```python
from build123d import *

# Parameters (mm, degrees)
BASE_BLOCK_SKETCH_W   = 70
BASE_BLOCK_SKETCH_H   = 30
BASE_BLOCK_DEPTH      = 20
HINGE_EAR_SKETCH_R    = 5
HINGE_EAR_DEPTH       = 10
SIDE_BLOCK_SKETCH_W   = 10
SIDE_BLOCK_SKETCH_H   = 10
SIDE_BLOCK_DEPTH      = 10
STOP_BLOCK_SKETCH_W   = 10
STOP_BLOCK_SKETCH_H   = 10
STOP_BLOCK_10MM_DEPTH = 10
ROD_SKETCH_R          = 2.5
ROD_30MM_DEPTH        = 30


with BuildPart() as part:
    # Base Block Sketch → Base Block (new body)
    with BuildSketch(Plane.XY):
        with Locations((35, 15)):
            Rectangle(BASE_BLOCK_SKETCH_W, BASE_BLOCK_SKETCH_H)
    extrude(amount=BASE_BLOCK_DEPTH)

    # Hinge Ear Sketch → Hinge Ear (add)
    with BuildSketch(Plane(origin=(0, 0, 0), x_dir=(0, 0, -1), z_dir=(1, 0, 0))):
        with BuildLine():
            Line((-20, 40), (-20, 30))
            Line((-20, 30), (0, 30))
            Line((0, 30), (0, 40))
            ThreePointArc((0, 40), (-10, 50), (-20, 40))
        make_face()
        with Locations((-10, 40)):
            Circle(HINGE_EAR_SKETCH_R, mode=Mode.SUBTRACT)
    hinge_ear = extrude(amount=HINGE_EAR_DEPTH)

    # Hinge Ear Mirror: Hinge Ear across plane
    add(hinge_ear.mirror(Plane(origin=(35, 0, 0), x_dir=(0, 0, 1), z_dir=(1, 0, 0))))

    # Side Block Sketch → Side Block (add)
    with BuildSketch(Plane.XY.offset(20)):
        with Locations((55, 15)):
            Rectangle(SIDE_BLOCK_SKETCH_W, SIDE_BLOCK_SKETCH_H)
    side_block = extrude(amount=SIDE_BLOCK_DEPTH)

    # Stop Block Sketch → Stop Block 10mm (add)
    with BuildSketch(Plane.XY.offset(20)):
        with Locations((15, 15)):
            Rectangle(STOP_BLOCK_SKETCH_W, STOP_BLOCK_SKETCH_H)
    stop_block_10mm = extrude(amount=STOP_BLOCK_10MM_DEPTH)

    # Rod Sketch → Rod 30mm (add)
    with BuildSketch(Plane(origin=(20, 0, 0), x_dir=(0, 0, -1), z_dir=(1, 0, 0))):
        with Locations(Location((-25, 15, 0), (0, 0, 180))):
            Circle(ROD_SKETCH_R)
    rod_30mm = extrude(amount=ROD_30MM_DEPTH)

    # Block and Rod Mirror: Side Block, Stop Block 10mm, Rod 30mm across plane
    add(side_block.mirror(Plane.XY.offset(10)))
    add(stop_block_10mm.mirror(Plane.XY.offset(10)))
    add(rod_30mm.mirror(Plane.XY.offset(10)))


solid = part.part
```
The model under review builds one solid part; all positions refer to its coordinate system, in mm. A direction names the side the tool comes from. Coordinates: 2 decimals unless noted, no trailing zeros. Order: outer loops, then holes, each group sorted by start corner. A loop starts at its lowest first (then second) coordinate and runs counter-clockwise, first axis right, second up. Notation, with made-up numbers: (35, -16) -> (44, -16) arc R25 ccw to (44, 17) -> close; hole circle Ø6 at (81, -33.75). An arc over 180 degrees is marked (long way). Answer in a Markdown table with one row per item. Add a question column.
Item 1: We need section B-B on x = 42. Write out the cut boundary in (y, z).
Item 2: Mouldability with a two-part tool opening along Z and no side actions: class faces 6 (the flat face through (55, 15, -10)), 7 (the cylindrical face through (5, 44, 7)), 8 (the flat face through (60, 38, 15)) as +Z half, -Z half, draft (parallel to the pull), parting line (faces both ways), or undercut.
Item 3: Machinability: for faces 1 (the flat face through (15, 20, 25)), 2 (the flat face through (60, 15, 25)), 3 (the flat face through (60, 15, -5)), 4 (the flat face through (55, 20, -5)), 5 (the flat face through (10, 15, 25)), which of the approach directions +Z, -Z, +X, -X, +Y, -Y give a long, thin tool a straight path to every point of the face, cutting with its end or side? Answer none if there is none.
Item 4: We need section D-D on y = 15. Write out the cut boundary in (x, z).
Item 5: We need section C-C on z = 10. Write out the cut boundary in (x, y).
Item 6: Clearance check with flat-ended pins moving along their axes: pin 1 (3 mm diameter, centred on x = 36.5, y = 6, fed in from -Z); pin 2 (2 mm diameter, centred on x = 50, y = 8, fed in from +Z); pin 3 (5 mm diameter, centred on x = 52.5, z = 24.5, fed in from +Y). State where each tip first meets the part, or that it passes through.
Item 7: To check wall thickness, follow probe 1 along Z at (x, y) = (22.5, 15); probe 2 along Y at (x, z) = (66, 10); probe 3 along X at (y, z) = (11.5, -6.5). State the ranges of each line that lie inside material, in increasing order.
Item 8: We need section A-A on z = 21.5. Write out the cut boundary in (x, y), plus the area to 3 significant figures.
Final values:
| question | item | result |
|---|---|---|
| 1 | outline | (0, 0) -> (30, 0) -> (30, 20) -> (0, 20) -> close; circle Ø5 at (15, -5); circle Ø5 at (15, 25) |
| 2 | face 6 | -Z half |
| 2 | face 7 | undercut |
| 2 | face 8 | draft |
| 3 | face 1 | +Z, +X, -X, +Y |
| 3 | face 2 | +Z, +X, +Y, -Y |
| 3 | face 3 | -Z, +X, +Y, -Y |
| 3 | face 4 | -Z, +X, -X, +Y |
| 3 | face 5 | +Z, -X, +Y, -Y |
| 4 | outline | (0, 0) -> (10, 0) -> (10, -10) -> (20, -10) -> (20, -7.5) -> (50, -7.5) -> (50, -10) -> (60, -10) -> (60, 0) -> (70, 0) -> (70, 20) -> (60, 20) -> (60, 30) -> (50, 30) -> (50, 27.5) -> (20, 27.5) -> (20, 30) -> (10, 30) -> (10, 20) -> (0, 20) -> close; hole (20, -2.5) -> (50, -2.5) -> (50, 0) -> (20, 0) -> close; hole (20, 20) -> (50, 20) -> (50, 22.5) -> (20, 22.5) -> close |
| 5 | outline | (0, 0) -> (70, 0) -> (70, 35) -> (60, 35) -> (60, 30) -> (10, 30) -> (10, 35) -> (0, 35) -> close; (0, 45) -> (10, 45) -> (10, 50) -> (0, 50) -> close; (60, 45) -> (70, 45) -> (70, 50) -> (60, 50) -> close |
| 6 | pin 1 | stops at z = 0 |
| 6 | pin 2 | stops at z = 20 |
| 6 | pin 3 | stops at y = 20 |
| 7 | probe 1 | z = -7.5 to -2.5, 0 to 20, 22.5 to 27.5 |
| 7 | probe 2 | y = 0 to 35, 45 to 50 |
| 7 | probe 3 | x = 10 to 20, 50 to 60 |
| 8 | outline | (10, 10) -> (20, 10) -> (20, 20) -> (10, 20) -> close; (50, 10) -> (60, 10) -> (60, 20) -> (50, 20) -> close |
| 8 | area | 200 mm2 |
